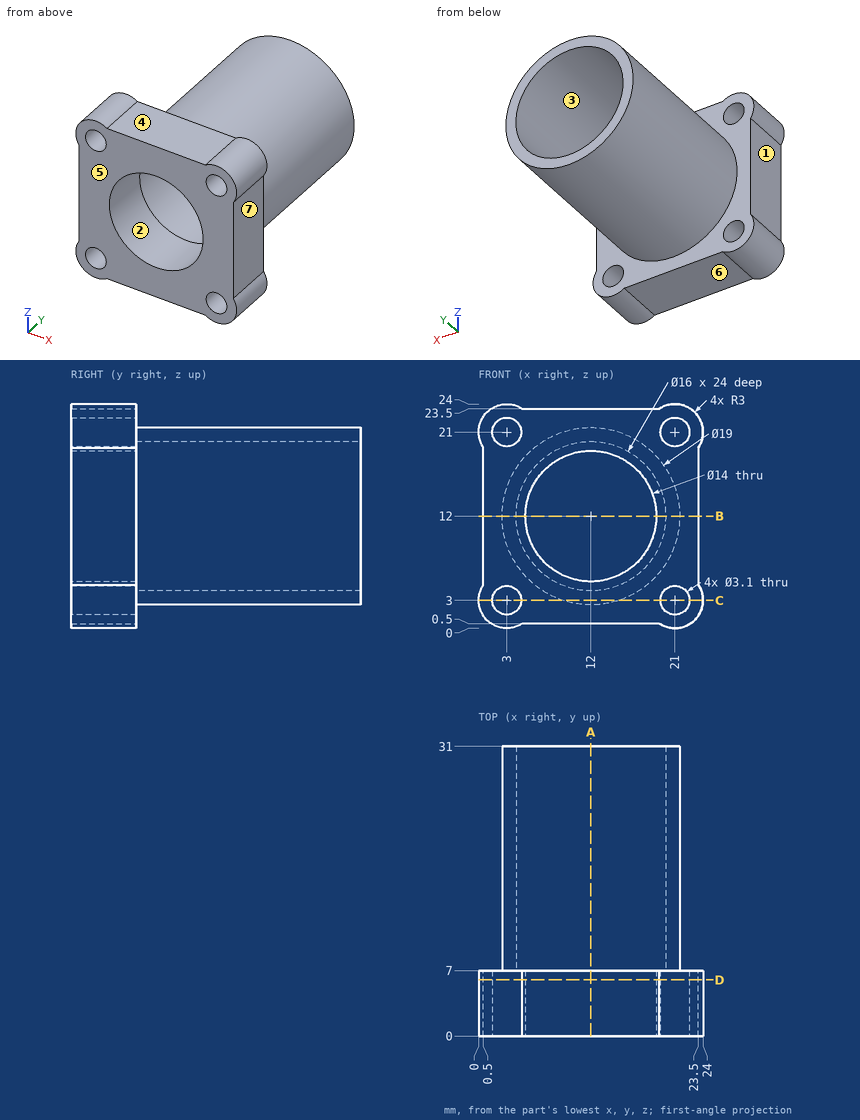
Study the drawing (mm; zero at the part's minimum x, y, z) and answer. A direction names the side the tool comes from. Give positions to 0.01 mm unless a question says otherwise; leave off trailing zeros. Write each loop counter-clockwise with the first axis right and the second up, starting at its lowest first coordinate (ties: lowest second). Pieces come first, ordered by that corner, then holes. Notation, with made-up numbers: M 18.5,37.5 L 49.5,37.5 A20 ccw 49.5,58.5 Z; hole C 48.5,32.5 d11. An arc over 180 degrees is marked long. Put each result on its own line as item: value. Start each with the question number.
1. Which of the six approach directions +Z, -Z, +X, -X, +Y, -Y give full straight-line access (tool end or side, diameter ignored) to the marked faces 1, 2, 3 and 4?
2. For a pull along X with two mould halves and no side action, classify the marked faces 5, 6 and 7 as released by +X, released by -X, zero draft, split by the parting line, or undercut.
3. Consider line 1 along X through (y, z) = (3.75, 21); line 2 along Y through (x, z) = (2.5, 15); line 3 along X through (y, z) = (16, 11.75). Determine where each line is inside the solid, lowest interval first.
4. The part is cut by section A-A, the plane x = 12. Give the vertices of the cut face in (y, z).
5. The part is cut by section B-B, the plane z = 12. Give the vertices of the cut face in (x, y).
6. The part is cut by section C-C, the plane z = 3. Give the vertices of the cut face in (x, y), and give its area (3 significant figures).
7. Each of these flat-tipped pins is pushed along its axis until it touches: pin 1 Ø12 at (x, y) = (7, 6) entering from -Z; pin 2 Ø3.5 at (y, z) = (5, 12.5) entering from +X; pin 3 Ø2 at (y, z) = (4.5, 11.5) entering from -X; pin 4 Ø8 at (x, z) = (14.5, 9) entering from +Y. Where does it stop, or does it pass through?
8. The part is cut by section D-D, the plane y = 6. Give the vertices of the cut face in (x, z).
Final values:
1. face 1: -X, +Y, -Y
1. face 2: +Y, -Y
1. face 3: +Y
1. face 4: +Z, +Y, -Y
2. face 5: zero draft
2. face 6: undercut
2. face 7: released by +X
3. line 1: x = 0 to 1.45, 4.55 to 19.45, 22.55 to 24
3. line 2: y = 0 to 7
3. line 3: x = 2.5 to 4, 20 to 21.5
4. outline: M 0,0.5 L 7,0.5 L 7,2.5 L 31,2.5 L 31,4 L 7,4 L 7,5 L 0,5 Z; M 0,19 L 7,19 L 7,20 L 31,20 L 31,21.5 L 7,21.5 L 7,23.5 L 0,23.5 Z
5. outline: M 0.5,0 L 5,0 L 5,7 L 4,7 L 4,31 L 2.5,31 L 2.5,7 L 0.5,7 Z; M 19,0 L 23.5,0 L 23.5,7 L 21.5,7 L 21.5,31 L 20,31 L 20,7 L 19,7 Z
6. outline: M 0,0 L 1.45,0 L 1.45,7 L 0,7 Z; M 4.55,0 L 19.45,0 L 19.45,7 L 15.04,7 L 15.04,31 L 8.96,31 L 8.96,7 L 4.55,7 Z; M 22.55,0 L 24,0 L 24,7 L 22.55,7 Z
6. area: 271 mm²
7. pin 1: stops at z = 0
7. pin 2: stops at x = 23.5
7. pin 3: stops at x = 0.5
7. pin 4: stops at y = 7
8. outline: M 0.5,4.66 A3 ccw 4.66,0.5 L 19.34,0.5 A3 ccw 23.5,4.66 L 23.5,19.34 A3 ccw 19.34,23.5 L 4.66,23.5 A3 ccw 0.5,19.34 Z; hole C 3,3 d3.1; hole C 3,21 d3.1; hole C 12,12 d14; hole C 21,3 d3.1; hole C 21,21 d3.1
